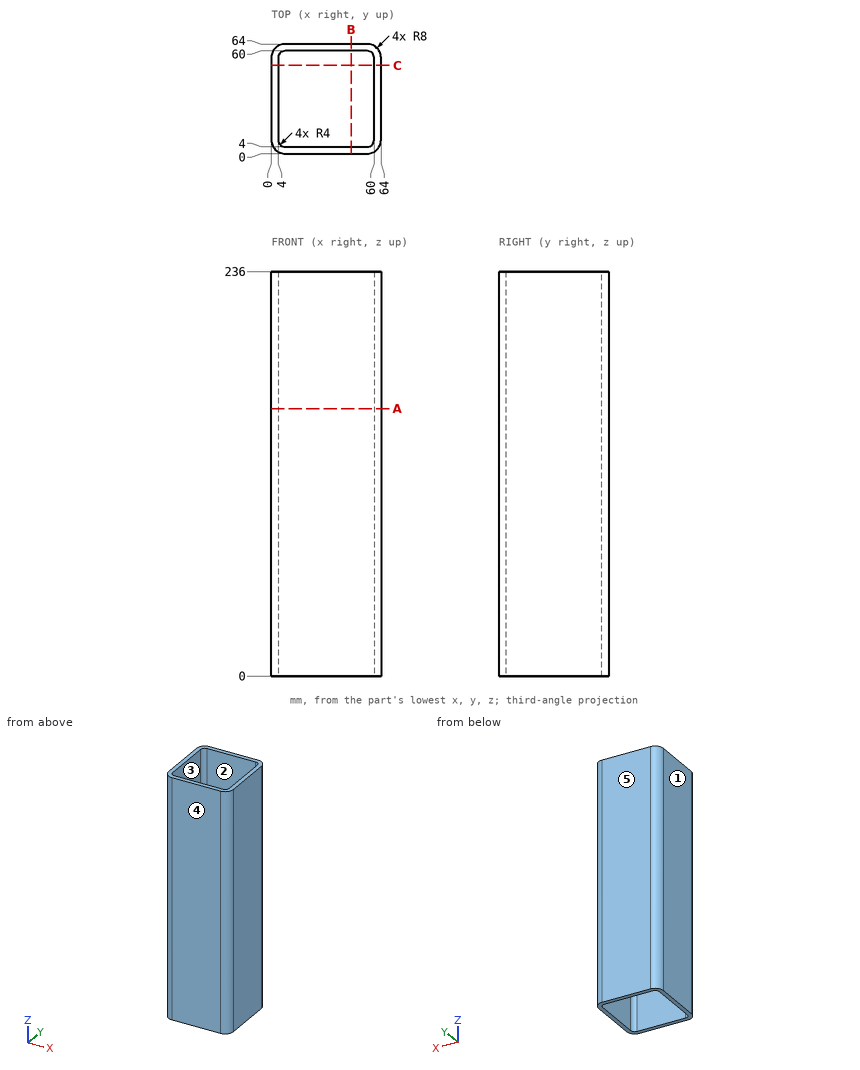
Source: three-view drawing plus pictorial views. Frame: mm from the lowest corner of the part. A direction names the side the tool comes from. Round coordinates to 2 decimals unless told otherwise and drop trailing zeros. Order: outer loops, then holes, each group sorted by start corner. A loop starts at its lowest first (then second) coordinate and runs counter-clockwise, first axis right, second up. Notation, with made-up numbers: (-31, -24.5) -> (-8, -24.5) arc R24 cw to (-8, 12.5) -> close; hole circle Ø7 at (63, 0.5). An arc over 180 degrees is marked (long way). Use CSV: the item, a comma, the result in double quotes. Start each with the question number.
1) Draft query along Y for the marked faces 3, 4 and 5. Return one class per face: +Y half, -Y half, draft (parallel to the pull), parting line (faces both ways), or undercut.
2) Section B-B (x = 46.5). Return the cut outline in (y, z).
3) Section A-A (z = 156). Return the cut outline in (x, y).
4) Set-up query: the marked faces 1 and 2. Return all of +Z, -Z, +X, -X, +Y, -Y with unobstructed straight access to the full face (end or side cutting, diameter ignored); none if empty.
5) Material intervals for line 1 along X through (y, z) = (40, 125); line 2 along Y through (x, z) = (61, 185) (3 decimals), sorted ascending. Write a range as from..to.
Returned:
1,face 3,"undercut"
1,face 4,"-Y half"
1,face 5,"+Y half"
2,outline,"(0, 0) -> (4, 0) -> (4, 236) -> (0, 236) -> close; (60, 0) -> (64, 0) -> (64, 236) -> (60, 236) -> close"
3,outline,"(0, 8) arc R8 ccw to (8, 0) -> (56, 0) arc R8 ccw to (64, 8) -> (64, 56) arc R8 ccw to (56, 64) -> (8, 64) arc R8 ccw to (0, 56) -> close; hole (4, 8) arc R4 ccw to (8, 4) -> (56, 4) arc R4 ccw to (60, 8) -> (60, 56) arc R4 ccw to (56, 60) -> (8, 60) arc R4 ccw to (4, 56) -> close"
4,face 1,"+Z, -Z, -X, +Y, -Y"
4,face 2,"+Z, -Z"
5,line 1,"x = 0..4, 60..64"
5,line 2,"y = 1.755..62.245"
